Can you work these out from the model? Positions are in its coordinate system, mm. A direction names the side the tool comes from. Give positions to 0.01 mm unless a question says otherwise; leave off trailing zeros. Write each loop counter-clockwise with the first axis right and the second up, starting at its lowest first coordinate (ties: lowest second). Pieces come first, ordered by that corner, then holes. Notation, with made-up numbers: (26, -0.5) - (81, -0.5) arc R22 cw to (81, 9.5) - close; hole circle Ø11 at (14, 63.5). An arc over 180 degrees is marked (long way). Use a Markdown table: item, result. Add a question column.
```python
from build123d import *

# Parameters (mm, degrees)
SKETCH_2_R                   = 1.25
CUT_EXTRUDE_1_DEPTH          = 32.559467676
HOLE_WIZARD_M4_1_D           = 3.3
HOLE_WIZARD_M4_1_CSINK_D     = 4.05
HOLE_WIZARD_M4_1_CSINK_ANGLE = 90
CHAMFER_1_SIZE               = 0.5
CHAMFER_2_SIZE               = 1
CUT_EXTRUDE_2_DEPTH          = 10
FILLET_1_R                   = 3
HOLE_WIZARD_M3_1_D           = 2.5


with BuildPart() as part:
    # 草图1 → 旋转1 (revolve)
    with BuildSketch(Plane(origin=(0, 0, 0), x_dir=(1, 0, 0), z_dir=(0, 1, 0)), mode=Mode.PRIVATE) as revolve_1_sk:
        Polygon((0, 7), (0, 16), (3, 16), (3, 10), (13, 10), (13, 9), (25, 9), (25, 7), (22, 7), (22, 0), (19, 0), (19, 7), align=None)
    revolve(revolve_1_sk.sketch.rotate(Axis((-407.867518885, 0, 0), (1, 0, 0)), 180), axis=Axis((-407.867518885, 0, 0), (1, 0, 0)))

    # 草图2 → 切除-拉伸1 (cut, through all)
    with BuildSketch(Plane(origin=(3, 0, 0), x_dir=(0, 0, -1), z_dir=(1, 0, 0))):
        with Locations((0, 13)):
            Circle(SKETCH_2_R)
        with Locations((13, 0)):
            Circle(SKETCH_2_R)
        with Locations((0, -13)):
            Circle(SKETCH_2_R)
        with Locations((-13, 0)):
            Circle(SKETCH_2_R)
    extrude(amount=-CUT_EXTRUDE_1_DEPTH, mode=Mode.SUBTRACT)

    # M4 螺纹孔1 (through all)
    with Locations(Plane(origin=(22, 0, 0), x_dir=(0, 0, -1), z_dir=(1, 0, 0))):
        with Locations((0, 0)):
            CounterSinkHole(HOLE_WIZARD_M4_1_D / 2, HOLE_WIZARD_M4_1_CSINK_D / 2, counter_sink_angle=HOLE_WIZARD_M4_1_CSINK_ANGLE)

    # 倒角1
    chamfer_1_edges = [part.edges().sort_by_distance(p)[0] for p in [
        (25, 0, -9),
        (13, 0, -10),
    ]]
    chamfer(chamfer_1_edges, length=CHAMFER_1_SIZE)

    # 倒角2
    chamfer_2_edges = [part.edges().sort_by_distance(p)[0] for p in [
        (0, 0, -7),
    ]]
    chamfer(chamfer_2_edges, length=CHAMFER_2_SIZE)

    # 草图5 → 切除-拉伸2 (cut)
    with BuildSketch(Plane(origin=(3, 0, 0), x_dir=(0, 0, -1), z_dir=(1, 0, 0))):
        with BuildLine():
            Line((1.001966601, 15.968596148), (15.968596148, 1.001966601))
            ThreePointArc((15.968596148, 1.001966601), (11.313708499, 11.313708499), (1.001966601, 15.968596148))
        make_face()
    extrude(amount=-CUT_EXTRUDE_2_DEPTH, mode=Mode.SUBTRACT)

    # 圆角1
    fillet_1_edges = [part.edges().sort_by_distance(p)[0] for p in [
        (1.5, 15.968596148, -1.001966601),
        (1.5, 1.001966601, -15.968596148),
    ]]
    fillet(fillet_1_edges, radius=FILLET_1_R)

    # M3 螺纹孔1 (through all)
    with Locations(Plane(origin=(3, 13, 0), x_dir=(0, 0, 1), z_dir=(1, 0, 0))):
        with Locations((0, 0), (13, 13), (0, 26), (-13, 13)):
            Hole(HOLE_WIZARD_M3_1_D / 2)


solid = part.part
```
Q1. I'm going to push flat-ended pins straight in: P1, Ø6, axis at x = 19, z = -11, coming from the -Y side; P2, Ø16, axis at y = 0, z = 0, coming from the +X side; P3, Ø1.5, axis at x = 3, y = -10, coming from the -Z side; P4, Ø4, axis at x = 7.5, y = 8.5, coming from the -Z side. Where does each tip first touch, or does it pass through?
Q2. Suppose I cut it at D-D (x = 6.5). Please give me the cut outline in (y, z), and give its area (3 significant figures).
Q3. On a 3-axis mill with a long thin cutter (end or side, diameter ignored), from which of +Z, -Z, +X, -X, +Y, -Y can I reach the whole of each face in a straight line? I mean faces 1 (the cylindrical face through (1.52, 14.24, 0.16)), 2 (the flat face through (19, -2, 0)), 3 (the cylindrical face through (8, 0, -10)). Say none if no direction works.
Q4. Suppose I cut it at A-A (x = 2.25). Please give me the cut outline in (y, z), and give its area (3 significant figures).
Q5. If I drill on probe 1 along Y at (x, z) = (10.75, 0); probe 2 along Y at (x, z) = (22.8, 0); probe 3 along X at (y, z) = (4.5, -2.5), over which ranges is the centre line in solid material (lowest first)? Write a range as [from, to].
Q6. Suppose I cut it at C-C (z = -13). Please give me the cut outline in (x, y), and give its area (3 significant figures).
Q7. If we mould it in two halves opening along Y, with no side actions, what happens to faces 4 (the flat face through (3, -0.2, 10.4)), 5 (the cylindrical face through (1.52, -11.76, 0.16)), 6 (the flat face through (1.52, 8.58, -8.39))? For each: released by +Y, released by -Y, zero draft, split by the parting line, or undercut.
Q8. Suppose I cut it at B-B (y = -13). Please give me the cut outline in (x, z).
Derived:
| question | item | result |
|---|---|---|
| 1 | P1 | y = -4.12 |
| 1 | P2 | x = 25 |
| 1 | P3 | z = -13.06 |
| 1 | P4 | z = -7.6 |
| 2 | outline | circle Ø20 at (0, 0); hole circle Ø14 at (0, 0) |
| 2 | area | 160 mm² |
| 3 | face 1 | +X, -X |
| 3 | face 2 | -X |
| 3 | face 3 | +X |
| 4 | outline | (-0.33, -16) arc R3 ccw to (1.85, -15.12) - (15.12, -1.85) arc R3 ccw to (16, 0.33) arc R16 ccw (long way) to start; hole circle Ø2.5 at (-13, 0); hole circle Ø14 at (0, 0); hole circle Ø2.5 at (0, -13); hole circle Ø2.5 at (0, 13); hole circle Ø2.5 at (13, 0) |
| 4 | area | 572 mm² |
| 5 | probe 1 | [-10, -7], [7, 10] |
| 5 | probe 2 | [-9, -7], [7, 9] |
| 5 | probe 3 | [19, 22] |
| 6 | outline | (0, -9.33) - (3, -9.33) - (3, -1.25) - (0, -1.25) - close; (0, 1.25) - (3, 1.25) - (3, 3.97) - (0, 3.97) - close |
| 6 | area | 32.4 mm² |
| 7 | face 4 | zero draft |
| 7 | face 5 | undercut |
| 7 | face 6 | released by +Y |
| 8 | outline | (0, -9.33) - (3, -9.33) - (3, -1.25) - (0, -1.25) - close; (0, 1.25) - (3, 1.25) - (3, 9.33) - (0, 9.33) - close |
